Can you work these out from the drawing? Everything is in mm from the part's minimum corner. Coordinates: 2 decimals unless noted, no trailing zeros. Order: outer loops, then holes, each group sorted by start corner. A loop starts at its lowest first (then second) coordinate and runs counter-clockwise, first axis right, second up. Notation, with made-up numbers: (61, -38.5) -> (68, -38.5) arc R31 cw to (68, -2.5) -> close; hole circle Ø2 at (30.5, -13.5). An arc over 180 degrees is marked (long way). Write item = value, one per line. Start each with the question number.
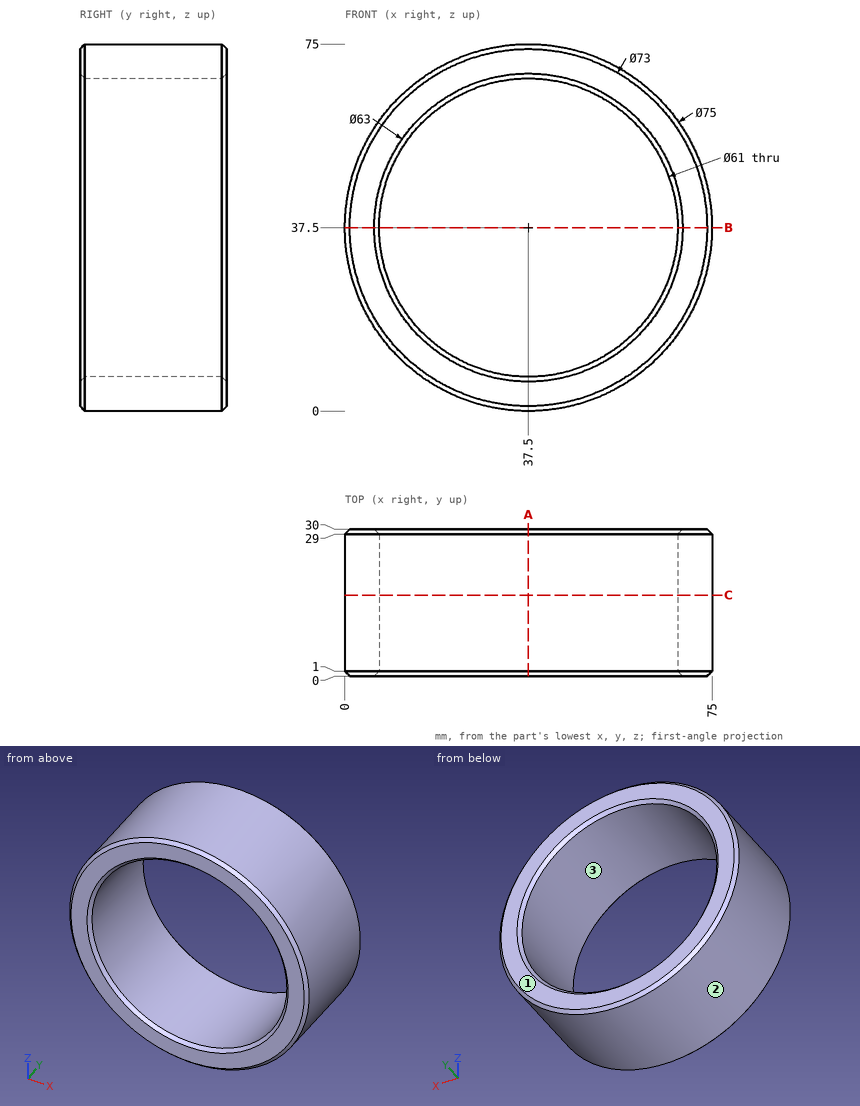
(1) Imagine slicing it at A-A (x = 37.5). Write out the boundary of the cut face in (y, z).
(2) Imagine slicing it at C-C (y = 16.5). Write out the boundary of the cut face in (x, z).
(3) If I drill on L1, parallel to X at y = 15.75, z = 37.5; L2, parallel to Z at x = 38.5, y = 13.5; L3, parallel to Z at x = 14, y = 3.75, over which ranges is the centre line in solid material (lowest first)? Write a range as from..to.
(4) Thinking about a two-plate mould opening in X: for the marked faces 1, 2 and 3, which applies, +X half, -X half, draft (parallel to the pull), parting line (faces both ways), or undercut?
(5) Imagine slicing it at B-B (z = 37.5). Write out the boundary of the cut face in (x, y).
(6) For P1, Ø1, axis at y = 20.5, z = 11.5, coming from the +X side; P2, Ø2, axis at y = 11, z = 42, coming from the +X side; P3, Ø6, axis at y = 8.5, z = 46, coming from the -X side, each with a flat end and sliding along its axis, tell me the tip position at first contact or that it passes through.
Result set:
q1.outline = (0, 1) -> (1, 0) -> (29, 0) -> (30, 1) -> (30, 6) -> (29, 7) -> (1, 7) -> (0, 6) -> close; (0, 69) -> (1, 68) -> (29, 68) -> (30, 69) -> (30, 74) -> (29, 75) -> (1, 75) -> (0, 74) -> close
q2.outline = circle Ø75 at (37.5, 37.5); hole circle Ø61 at (37.5, 37.5)
q3.L1 = 0..7, 68..75
q3.L2 = 0.01..7.02, 67.98..74.99
q3.L3 = 8.28..18.06, 56.94..66.72
q4.face_1 = draft
q4.face_2 = parting line
q4.face_3 = undercut
q5.outline = (0, 1) -> (1, 0) -> (6, 0) -> (7, 1) -> (7, 29) -> (6, 30) -> (1, 30) -> (0, 29) -> close; (68, 1) -> (69, 0) -> (74, 0) -> (75, 1) -> (75, 29) -> (74, 30) -> (69, 30) -> (68, 29) -> close
q6.P1 = 65
q6.P2 = 74.84
q6.P3 = 0.41
